Design review of the part built by this model. Coordinates are the model's own, in mm. Face numbers are marked on the shaded views. A direction names the side the tool comes from. Coordinates: 2 decimals unless noted, no trailing zeros. Write each loop counter-clockwise with the first axis right and the second up, starting at its lowest first coordinate (ties: lowest second). Pieces come first, ordered by that corner, then holes.
Q1. Add section C-C, the plane y = 94.5. Give the boundary of the cut face in (x, z).
Q2. Add section D-D, the plane z = 342.5. Give the boundary of the cut face in (x, y).
Q3. To check wall thickness, follow probe 1 along Y at (x, z) = (97.5, 375.5); probe 2 along X at (y, z) = (123.2, 50). State the ranges of each line that lie inside material, in increasing order.
Q4. Machinability: for the marked faces 5 and 6, which of the approach directions +Z, -Z, +X, -X, +Y, -Y give a long, thin tool a straight path to every point of the face, cutting with its end or side? Answer none if there is none.
Q5. Clearance check with a flat-ended pin moving along its axis: pin 1 Ø21.5 at (x, z) = (63, 50) entering from +Y. State where the tip first meets the part, or that it passes through.
Q6. Add section A-A, the plane z = 50. Give the boundary of the cut face in (x, y).
Q7. The part is to be moulded in two halves that separate along Y. For the marked faces 1, 2, 3 and 4, say which applies: +Y half, -Y half, draft (parallel to the pull), parting line (faces both ways), or undercut.
Q8. Add section B-B, the plane x = 63. Give the boundary of the cut face in (y, z), plus the area to 3 significant figures.
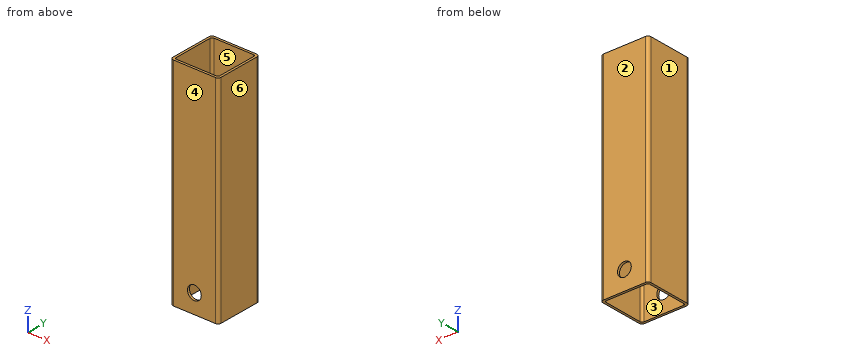
from build123d import *

# Parameters (mm, degrees)
SKETCH1_W           = 126
SKETCH1_H           = 126
SKETCH1_W_2         = 114
SKETCH1_H_2         = 114
BOSS_EXTRUDE1_DEPTH = 560
FILLET1_R           = 8
FILLET2_R           = 5
SKETCH3_R           = 18
CUT_EXTRUDE1_DEPTH  = 260


with BuildPart() as part:
    # Sketch1 → Boss-Extrude1 (new body)
    with BuildSketch(Plane.XY):
        with Locations((63, 63)):
            Rectangle(SKETCH1_W, SKETCH1_H)
        with Locations((63, 63)):
            Rectangle(SKETCH1_W_2, SKETCH1_H_2, mode=Mode.SUBTRACT)
    extrude(amount=BOSS_EXTRUDE1_DEPTH)

    # Fillet1
    fillet1_edges = [part.edges().sort_by_distance(p)[0] for p in [
        (0, 126, 280),
        (126, 126, 280),
        (126, 0, 280),
        (0, 0, 280),
    ]]
    fillet(fillet1_edges, radius=FILLET1_R)

    # Fillet2
    fillet2_edges = [part.edges().sort_by_distance(p)[0] for p in [
        (6, 120, 280),
        (6, 6, 280),
        (120, 6, 280),
        (120, 120, 280),
    ]]
    fillet(fillet2_edges, radius=FILLET2_R)

    # Sketch3 → Cut-Extrude1 (cut)
    with BuildSketch(Plane.XZ):
        with Locations(Location((63, 50, 0), (0, 0, 270))):
            Circle(SKETCH3_R)
    extrude(amount=-CUT_EXTRUDE1_DEPTH, mode=Mode.SUBTRACT)


solid = part.part
Here are the results:
1. outline: (0, 0) - (6, 0) - (6, 560) - (0, 560) - close; (120, 0) - (126, 0) - (126, 560) - (120, 560) - close
2. outline: (0, 8) arc R8 ccw to (8, 0) - (118, 0) arc R8 ccw to (126, 8) - (126, 118) arc R8 ccw to (118, 126) - (8, 126) arc R8 ccw to (0, 118) - close; hole (6, 11) arc R5 ccw to (11, 6) - (115, 6) arc R5 ccw to (120, 11) - (120, 115) arc R5 ccw to (115, 120) - (11, 120) arc R5 ccw to (6, 115) - close
3. probe 1: y = 0 to 6, 120 to 126
3. probe 2: x = 1.92 to 45, 81 to 124.08
4. face 5: +Z, -Z
4. face 6: +Z, -Z, +X, +Y, -Y
5. pin 1: passes through
6. outline: (0, 8) arc R8 ccw to (8, 0) - (45, 0) - (45, 6) - (11, 6) arc R5 cw to (6, 11) - (6, 115) arc R5 cw to (11, 120) - (45, 120) - (45, 126) - (8, 126) arc R8 ccw to (0, 118) - close; (81, 0) - (118, 0) arc R8 ccw to (126, 8) - (126, 118) arc R8 ccw to (118, 126) - (81, 126) - (81, 120) - (115, 120) arc R5 cw to (120, 115) - (120, 11) arc R5 cw to (115, 6) - (81, 6) - close
7. face 1: draft
7. face 2: +Y half
7. face 3: undercut
7. face 4: -Y half
8. outline: (0, 0) - (6, 0) - (6, 32) - (0, 32) - close; (0, 68) - (6, 68) - (6, 560) - (0, 560) - close; (120, 0) - (126, 0) - (126, 32) - (120, 32) - close; (120, 68) - (126, 68) - (126, 560) - (120, 560) - close
8. area: 6,290 mm2
